Part model, mm, in its own coordinate system. Face numbers are marked on the shaded views. A direction names the side the tool comes from. Give positions to 0.01 mm unless a question says otherwise; leave off trailing zeros. Write each loop counter-clockwise with the first axis right and the second up, starting at its lowest first coordinate (ties: lowest second). Pieces come first, ordered by that corner, then holes.
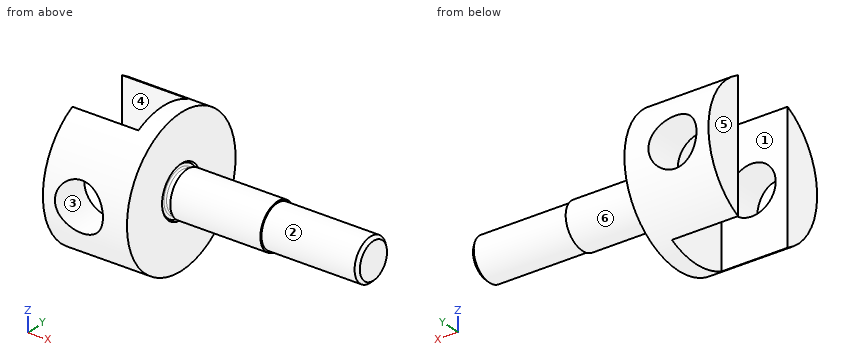
from build123d import *

# Parameters (mm, degrees)
SKETCH2_W               = 84.798069866
SKETCH2_H               = 22
CUT_EXTRUDE1_DEPTH      = 22
CUT_EXTRUDE2_DEPTH      = 51
CUT_EXTRUDE2_DEPTH_BACK = 22
SKETCH3_R               = 8
CHAMFER1_SIZE           = 1


with BuildPart() as part:
    # Sketch1 → Revolve1 (revolve)
    with BuildSketch(Plane.XY, mode=Mode.PRIVATE) as revolve1_sk:
        Polygon((0, 0), (0, 24), (28, 24), (28, 7), (30, 7), (30, 7.5), (60, 7.5), (60, 7), (92, 7), (92, 0), align=None)
    revolve(revolve1_sk.sketch.rotate(Axis((-36.181818182, 0, 0), (1, 0, 0)), 90), axis=Axis((-36.181818182, 0, 0), (1, 0, 0)))

    # Sketch2 → Cut-Extrude1 (cut)
    with BuildSketch(Plane.ZY):
        Rectangle(SKETCH2_W, SKETCH2_H)
    extrude(amount=-CUT_EXTRUDE1_DEPTH, mode=Mode.SUBTRACT)

    # Sketch3 → Cut-Extrude2 (cut, two sides: drawn at the far end of the back side and taken through both)
    with BuildSketch(Plane(origin=(0, -11, 0), x_dir=(1, 0, 0), z_dir=(0, 1, 0)).offset(-CUT_EXTRUDE2_DEPTH_BACK)):
        with Locations(Location((12, 0, 0), (0, 0, 90))):
            Circle(SKETCH3_R)
    extrude(amount=CUT_EXTRUDE2_DEPTH + CUT_EXTRUDE2_DEPTH_BACK, mode=Mode.SUBTRACT)

    # Sketch7 → Cut-Revolve1 (revolve, cut)
    with BuildSketch(Plane(origin=(0, 0, 0), x_dir=(1, 0, 0), z_dir=(0, 1, 0))):
        with BuildLine():
            Line((28, -6.5), (29.5, -6.5))
            Line((29.5, -6.5), (30, -7))
            Line((30, -7), (28, -7))
            Line((28, -7), (28, -8.5))
            Line((28, -8.5), (27.5, -8))
            Line((27.5, -8), (27.5, -7))
            ThreePointArc((27.5, -7), (27.646446609, -6.646446609), (28, -6.5))
        make_face()
    revolve(axis=Axis((0, 0, 0), (1, 0, 0)), mode=Mode.SUBTRACT)

    # Chamfer1
    chamfer1_edges = [part.edges().sort_by_distance(p)[0] for p in [
        (92, 0, -7),
    ]]
    chamfer(chamfer1_edges, length=CHAMFER1_SIZE)


solid = part.part
1) Saw through at B-B (z = 0). State how many separate pieces and enclosed holes the cut face has, and give its area (3 significant figures).
Check result:
separate pieces: 3
enclosed holes: 0
area: 1,370 mm2
2) Saw through at D-D (z = 11). Write the cut outline in (x, y), and give its area (3 significant figures).
Check result:
outline: (0, -21.33) - (28, -21.33) - (28, 21.33) - (0, 21.33) - (0, 11) - (22, 11) - (22, -11) - (0, -11) - close
area: 711 mm2
3) Flat gauge pins, fed straight in: P1, Ø8, axis at x = 67.5, z = -6, coming from the -Y side; P2, Ø10, axis at x = 16.5, z = 7, coming from the -Y side; P3, Ø1.5, axis at y = 15.5, z = -6, coming from the +X side; P4, Ø9.5, axis at x = 12, z = 0, coming from the +Y side. Where does each tip first touch, or does it go through?
Check result:
P1: stops at y = -6.71
P2: stops at y = -23.82
P3: stops at x = 28
P4: passes through
4) 3-axis set-ups, long thin cutter, end or side, ignore diameter. For the marked faces 4, 5 and 6: which of +Z, -Z, +X, -X, +Y, -Y reach the whole face in a straight line?
Check result:
face 4: +Z, -Z, -X
face 5: +Z, -Z, -X, +Y, -Y
face 6: +X
5) Drill centre lines: L1, parallel to X at y = 19, z = 0; L2, parallel to X at y = -15, z = 3; L3, parallel to X at y = -14, z = -13. Where is each one in solid material? Low to high.
Check result:
L1: x = 0 to 4, 20 to 28
L2: x = 0 to 4.58, 19.42 to 28
L3: x = 0 to 28
6) Saw through at C-C (y = -13). Write the cut outline in (x, z), and give its area (3 significant figures).
Check result:
outline: (0, -20.17) - (28, -20.17) - (28, 20.17) - (0, 20.17) - close; hole circle Ø16 at (12, 0)
area: 929 mm2
7) Mould opens along Z. For the marked faces 1, 2 and 3 say: +Z half, -Z half, draft (parallel to the pull), parting line (faces both ways), or undercut.
Check result:
face 1: draft
face 2: parting line
face 3: undercut
8) Saw through at A-A (x = 12). Write the cut outline in (y, z), and give its area (3 significant figures).
Check result:
outline: (-22.63, -8) arc R24 ccw to (-11, -21.33) - (-11, -8) - close; (-22.63, 8) - (-11, 8) - (-11, 21.33) arc R24 ccw to start; (11, -21.33) arc R24 ccw to (22.63, -8) - (11, -8) - close; (11, 8) - (22.63, 8) arc R24 ccw to (11, 21.33) - close
area: 390 mm2
